Part print with two shaded views. Sizes in mm from the minimum x, y, z corner. A direction names the side the tool comes from. Coordinates: 2 decimals unless noted, no trailing zeros. Loops run counter-clockwise (first coordinate to the right, second up) from the corner with the lowest first, then second, coordinate; pieces in that order, holes last.
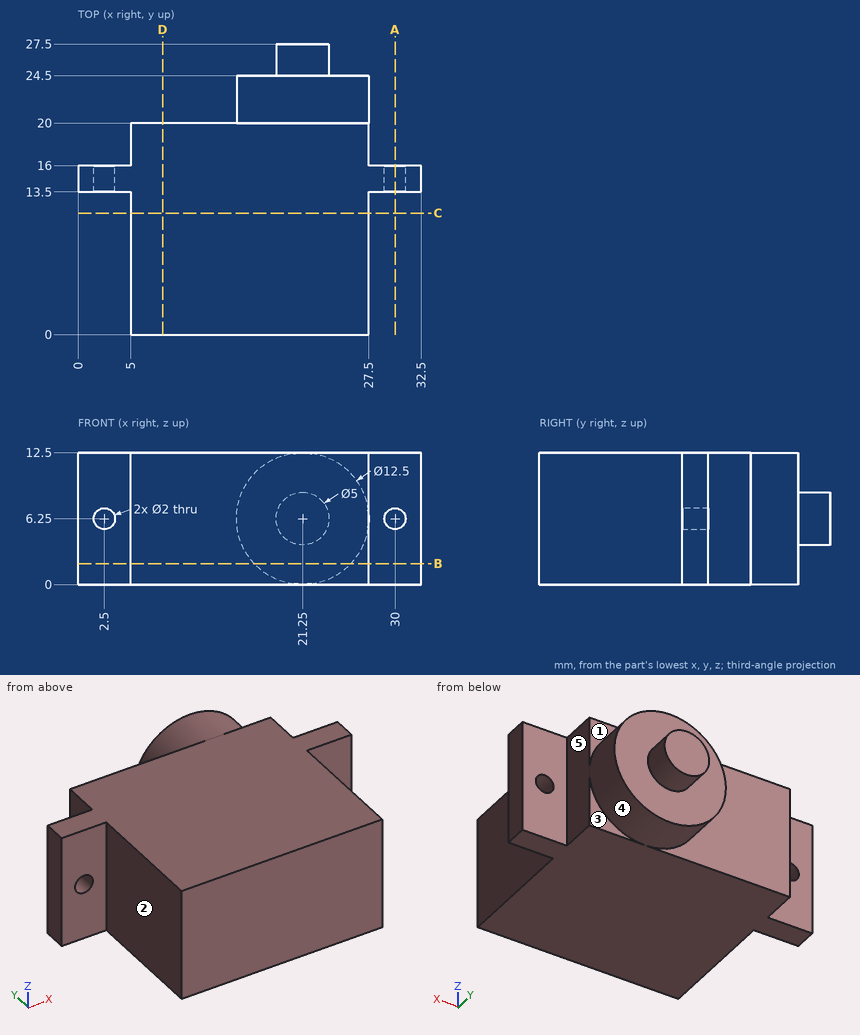
Q1. Slice it at C-C (y = 11.5). List the corners of the cut face in (x, z), and give its area (3 significant figures).
Answers:
outline: (5, 0) - (27.5, 0) - (27.5, 12.5) - (5, 12.5) - close
area: 281 mm2
Q2. Slice it at D-D (x = 8). List the corners of the cut face in (y, z), and give its area (3 significant figures).
Answers:
outline: (0, 0) - (20, 0) - (20, 12.5) - (0, 12.5) - close
area: 250 mm2
Q3. Slice it at B-B (z = 2). List the corners of the cut face in (x, y).
Answers:
outline: (0, 13.5) - (5, 13.5) - (5, 0) - (27.5, 0) - (27.5, 13.5) - (32.5, 13.5) - (32.5, 16) - (27.5, 16) - (27.5, 20) - (25.83, 20) - (25.83, 24.5) - (16.67, 24.5) - (16.67, 20) - (5, 20) - (5, 16) - (0, 16) - close
Q4. Drill centre lines: line 1 (X direction, y = 14.1, z = 6.25); line 2 (X direction, y = 6, z = 6.5); line 3 (Y direction, x = 7, z = 7.5). Where is each one in solid material? Low to high.
Answers:
line 1: x = 0 to 1.5, 3.5 to 29, 31 to 32.5
line 2: x = 5 to 27.5
line 3: y = 0 to 20
Q5. Which spindle directions (+Z, -Z, +X, -X, +Y, -Y) get a long thin tool onto all of the face, cutting with end or side? Do the marked faces 1, 2, 3, 4 and 5. Say none if no direction does.
Answers:
face 1: +Z, +X, +Y
face 2: +Z, -Z, -X, -Y
face 3: -Z, +X, +Y
face 4: +Y
face 5: +Z, -Z, +X, +Y
Q6. Slice it at A-A (x = 30). List the corners of the cut face in (y, z).
Answers:
outline: (13.5, 0) - (16, 0) - (16, 5.25) - (13.5, 5.25) - close; (13.5, 7.25) - (16, 7.25) - (16, 12.5) - (13.5, 12.5) - close
Q7. Flat gauge pins, fed straight in: P1, Ø1.5, axis at x = 30, z = 9, coming from the +Y side; P2, Ø6, axis at y = 21.5, z = 2, coming from the +X side; P3, Ø5.5, axis at x = 3, z = 8, coming from the +Y side. Where does each tip first touch, or does it go through?
Answers:
P1: stops at y = 16
P2: stops at x = 27.5
P3: stops at y = 20
